Geometry check sheet. Reference: drawing and pictorial views, mm from the part's lowest x, y, z. A direction names the side the tool comes from. Round coordinates to 2 decimals unless told otherwise and drop trailing zeros. Loops run counter-clockwise (first coordinate to the right, second up) from the corner with the lowest first, then second, coordinate; pieces in that order, holes last. Notation, with made-up numbers: (-15.75, 84.5) -> (22.25, 84.5) arc R24 ccw to (22.25, 100.5) -> close; hole circle Ø8 at (41, -26.75). An arc over 180 degrees is marked (long way). Use one line per item in the form item = value. Start each with the question number.
(1) Go/stop test with flat-tipped pins: pin 1 (4 mm diameter, centred on x = 3.5, y = 7, fed in from +Z); pin 2 (4 mm diameter, centred on y = 12.5, z = 14.5, fed in from +X); pin 3 (2 mm diameter, centred on x = 19.5, y = 4.5, fed in from +Z) (1 decimal). Record where each tip stops, or that it passes through.
(2) Set-up check for the marked faces 1, 2 and 3: record each of +Z, -Z, +X, -X, +Y, -Y from which the full face is reachable in a straight line by a thin tool's end or side.
(3) Sectioned sample at A-A (x = 22.5). Record the cut outline in (y, z).
(4) Material ranges on probe 1 along X at (y, z) = (11, 6); probe 2 along X at (y, z) = (2.5, 6.75); probe 3 along Z at (x, y) = (18, 6.5) (1 decimal), recorded low to high. Write a range as [from, to].
(5) Sectioned sample at C-C (y = 4). Record the cut outline in (x, z).
(6) Sectioned sample at B-B (z = 9.75). Record the cut outline in (x, y), and give its area (3 significant figures).
(7) Sectioned sample at D-D (x = 30). Record the cut outline in (y, z).
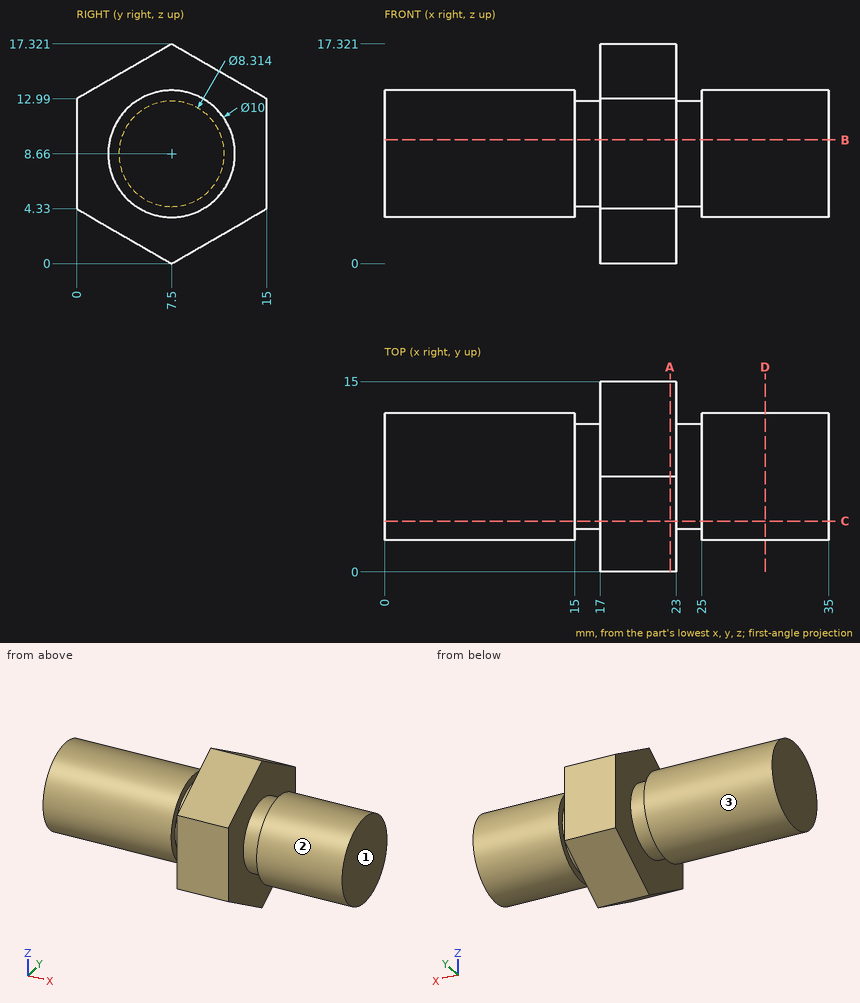
Checks:
q1.pin_1 = 13.66
q1.pin_2 = 23
q1.pin_3 = 16.2
q2.face_1 = +Z, -Z, +X, +Y, -Y
q2.face_2 = +X
q2.face_3 = -X
q3.outline = (0, 4.33) -> (7.5, 0) -> (15, 4.33) -> (15, 12.99) -> (7.5, 17.32) -> (0, 12.99) -> close
q4.probe_1 = [0, 15], [17, 23], [25, 35]
q4.probe_2 = [17, 23]
q4.probe_3 = [0.6, 16.7]
q5.outline = (0, 5.09) -> (15, 5.09) -> (15, 6.42) -> (17, 6.42) -> (17, 2.02) -> (23, 2.02) -> (23, 6.42) -> (25, 6.42) -> (25, 5.09) -> (35, 5.09) -> (35, 12.23) -> (25, 12.23) -> (25, 10.9) -> (23, 10.9) -> (23, 15.3) -> (17, 15.3) -> (17, 10.9) -> (15, 10.9) -> (15, 12.23) -> (0, 12.23) -> close
q6.outline = (0, 2.62) -> (15, 2.62) -> (15, 3.49) -> (17, 3.49) -> (17, 0) -> (23, 0) -> (23, 3.49) -> (25, 3.49) -> (25, 2.62) -> (35, 2.62) -> (35, 12.38) -> (25, 12.38) -> (25, 11.51) -> (23, 11.51) -> (23, 15) -> (17, 15) -> (17, 11.51) -> (15, 11.51) -> (15, 12.38) -> (0, 12.38) -> close
q6.area = 366 mm2
q7.outline = circle Ø10 at (7.5, 8.66)
